Could you check a few things on this drawing? It's one solid part, dimensions in mm from its lowest x, y, z. Give positions to 0.01 mm unless a question says otherwise; leave off trailing zeros. Order: outer loops, then holes, each group sorted by start corner. A loop starts at its lowest first (then second) coordinate and runs counter-clockwise, first axis right, second up.
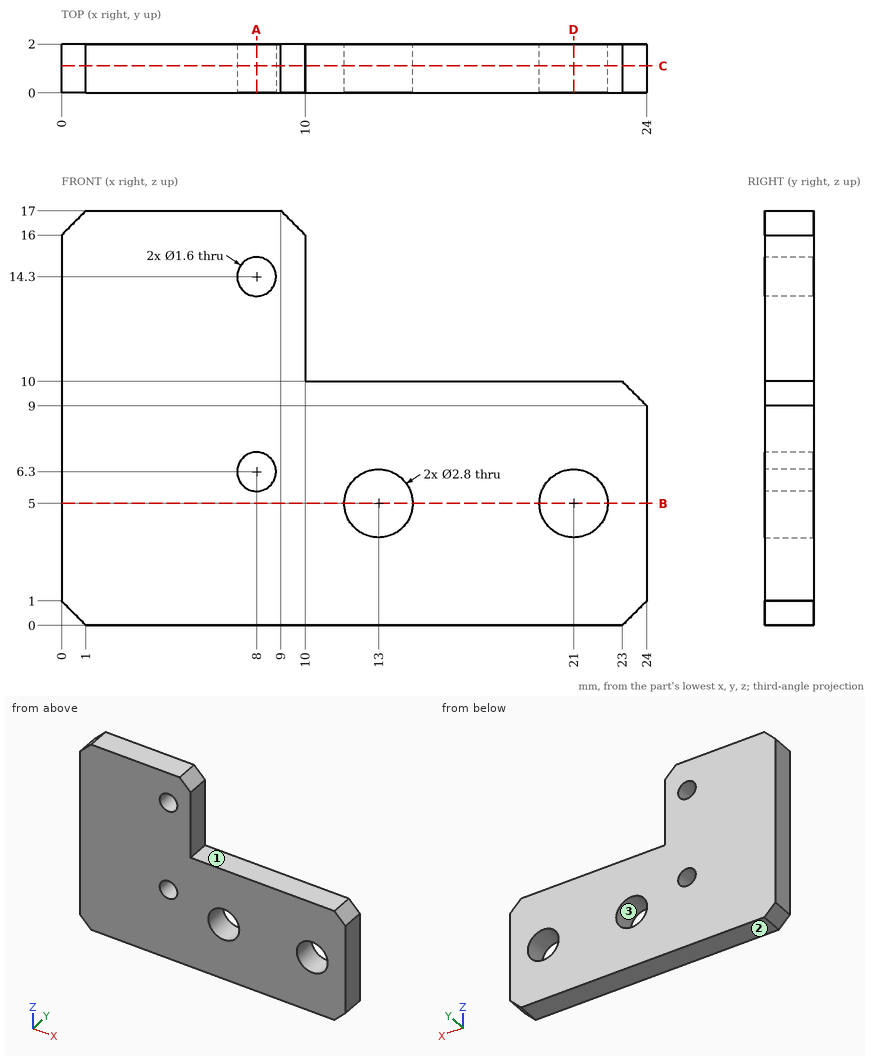
Item 1: Imagine slicing it at B-B on z = 5. List the corners of the cut face in (x, y) for me.
Findings:
outline: (0, 0) - (11.6, 0) - (11.6, 2) - (0, 2) - close; (14.4, 0) - (19.6, 0) - (19.6, 2) - (14.4, 2) - close; (22.4, 0) - (24, 0) - (24, 2) - (22.4, 2) - close
Item 2: We'd pull the mould along Z, two halves only. Please class the marked faces 1, 2 and 3: +Z half, -Z half, draft (parallel to the pull), parting line (faces both ways), or undercut.
Findings:
face 1: +Z half
face 2: -Z half
face 3: undercut
Item 3: Imagine slicing it at D-D on x = 21. List the corners of the cut face in (y, z) for me, then the cut area to 3 significant figures.
Findings:
outline: (0, 0) - (2, 0) - (2, 3.6) - (0, 3.6) - close; (0, 6.4) - (2, 6.4) - (2, 10) - (0, 10) - close
area: 14.4 mm2
Item 4: Please list where these lines run through material, in increasing order: line 1 along Z through (x, y) = (8, 1.1); line 2 along X through (y, z) = (0.4, 5); line 3 along X through (y, z) = (0.35, 4.25).
Findings:
line 1: z = 0 to 5.5, 7.1 to 13.5, 15.1 to 17
line 2: x = 0 to 11.6, 14.4 to 19.6, 22.4 to 24
line 3: x = 0 to 11.82, 14.18 to 19.82, 22.18 to 24
Item 5: For pin 1 (1.7 mm diameter, centred on x = 13, z = 5, fed in from -Y), with a flat end and sliding along its axis, tell me the tip position at first contact or that it passes through.
Findings:
pin 1: passes through
Item 6: Imagine slicing it at C-C on y = 1.1. List the corners of the cut face in (x, z) for me, then the cut area to 3 significant figures.
Findings:
outline: (0, 1) - (1, 0) - (23, 0) - (24, 1) - (24, 9) - (23, 10) - (10, 10) - (10, 16) - (9, 17) - (1, 17) - (0, 16) - close; hole circle Ø1.6 at (8, 6.3); hole circle Ø1.6 at (8, 14.3); hole circle Ø2.8 at (13, 5); hole circle Ø2.8 at (21, 5)
area: 291 mm2
Item 7: Imagine slicing it at A-A on x = 8. List the corners of the cut face in (y, z) for me, then the cut area to 3 significant figures.
Findings:
outline: (0, 0) - (2, 0) - (2, 5.5) - (0, 5.5) - close; (0, 7.1) - (2, 7.1) - (2, 13.5) - (0, 13.5) - close; (0, 15.1) - (2, 15.1) - (2, 17) - (0, 17) - close
area: 27.6 mm2
